from build123d import *

# Parameters (mm, degrees)
SKETCH2_R           = 6
BOSS_EXTRUDE1_DEPTH = 10


with BuildPart() as part:
    # Sketch2 → Boss-Extrude1 (new body)
    with BuildSketch(Plane.XY.offset(-10)):
        with BuildLine():
            Line((70, 40), (70, -79.604289692))
            ThreePointArc((70, -79.604289692), (85, -94.604289692), (100, -79.604289692))
            Line((100, -79.604289692), (100, 40))
            ThreePointArc((100, 40), (85, 55), (70, 40))
        make_face()
        with Locations((85, 40)):
            Circle(SKETCH2_R, mode=Mode.SUBTRACT)
        with Locations((85, -79.604289692)):
            Circle(SKETCH2_R, mode=Mode.SUBTRACT)
    extrude(amount=BOSS_EXTRUDE1_DEPTH)


solid = part.part
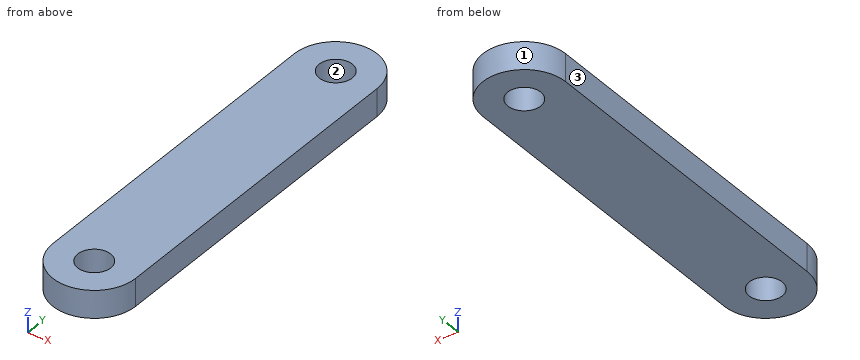
The model under review builds one solid part; all positions refer to its coordinate system, in mm. Face numbers are marked on the shaded views. Round coordinates to 2 decimals unless told otherwise and drop trailing zeros. Loops run counter-clockwise (first coordinate to the right, second up) from the corner with the lowest first, then second, coordinate; pieces in that order, holes last. Notation, with made-up numbers: M -40,29.25 L -33,29.25 A23 cw -33,61.25 Z; hole C 57,20 d4. An arc over 180 degrees is marked long. Answer as a JSON object with one key per item and string values.
Item 1: The part is to be moulded in two halves that separate along Y. For the marked faces 1, 2 and 3, say which applies: +Y half, -Y half, draft (parallel to the pull), parting line (faces both ways), or undercut.
Check sheet entries:
{"face 1": "+Y half", "face 2": "undercut", "face 3": "draft"}
Item 2: We need section A-A, the plane z = -4.5. State the section outline as (x, y) points, and give its area (3 significant figures).
Check sheet entries:
{"outline": "M 70,-79.6 A15 ccw 100,-79.6 L 100,40 A15 ccw 70,40 Z; hole C 85,-79.6 d12; hole C 85,40 d12", "area": "4,070 mm2"}
Item 3: We need section C-C, the plane y = 42. State the section outline as (x, z) points, and give its area (3 significant figures).
Check sheet entries:
{"outline": "M 70.13,-10 L 79.34,-10 L 79.34,0 L 70.13,0 Z; M 90.66,-10 L 99.87,-10 L 99.87,0 L 90.66,0 Z", "area": "184 mm2"}
Item 4: We need section D-D, the plane x = 95.5. State the section outline as (y, z) points.
Check sheet entries:
{"outline": "M -90.32,-10 L 50.71,-10 L 50.71,0 L -90.32,0 Z"}
Item 5: Clearance check with a flat-ended pin moving along its axis: P1, Ø6, axis at x = 95, z = -3.5, coming from the +Y side. State where the tip first meets the part, or that it passes through.
Check sheet entries:
{"P1": "y = 53.27"}
Item 6: For line 1 along Y through (x, z) = (85, -7.5); line 2 along Y through (x, z) = (82, -4.5); line 3 along Y through (x, z) = (73.25, -1), list the stretches that pass through material, from the lowest coordinate up.
Check sheet entries:
{"line 1": "-94.6 to -85.6, -73.6 to 34, 46 to 55", "line 2": "-94.3 to -84.8, -74.41 to 34.8, 45.2 to 54.7", "line 3": "-88.93 to 49.32"}
Item 7: We need section B-B, the plane x = 85. State the section outline as (y, z) points, and give its area (3 significant figures).
Check sheet entries:
{"outline": "M -94.6,-10 L -85.6,-10 L -85.6,0 L -94.6,0 Z; M -73.6,-10 L 34,-10 L 34,0 L -73.6,0 Z; M 46,-10 L 55,-10 L 55,0 L 46,0 Z", "area": "1,260 mm2"}
